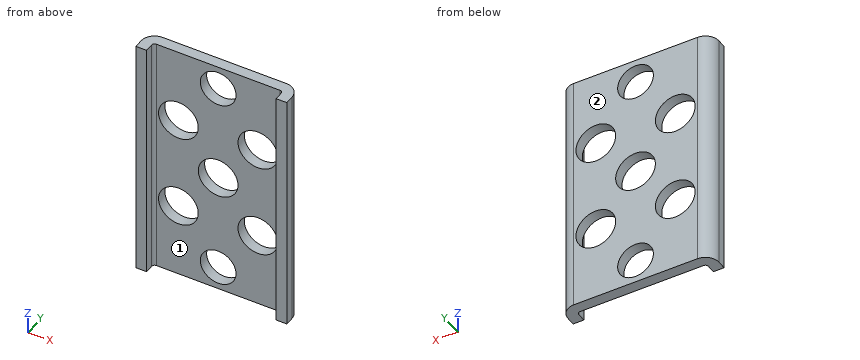
```python
from build123d import *

# Parameters (mm, degrees)
SKETCH1_W                      = 37.995749454
SKETCH1_H                      = 62
BOSS_EXTRUDE1_DEPTH            = 5.594860996
SKETCH2_W                      = 32.595749454
SKETCH2_H                      = 2.894860996
CUT_EXTRUDE1_DEPTH             = 66.086263633
F_10_0_10_DIAMETER_HOLE1_D     = 10
F_10_0_10_DIAMETER_HOLE1_DEPTH = 5.594860996
F_9_0_9_DIAMETER_HOLE1_D       = 9
F_9_0_9_DIAMETER_HOLE1_DEPTH   = 5.594860996
FILLET1_R                      = 0.7366
FILLET2_R                      = 3.4366


with BuildPart() as part:
    # Sketch1 → Boss-Extrude1 (new body)
    with BuildSketch(Plane(origin=(0, 0, 0), x_dir=(1, 0, 0), z_dir=(0, 1, 0))):
        with Locations((0, 45)):
            Rectangle(SKETCH1_W, SKETCH1_H)
    extrude(amount=-BOSS_EXTRUDE1_DEPTH)

    # Sketch2 → Cut-Extrude1 (cut, through all)
    with BuildSketch(Plane(origin=(0, 0, -76), x_dir=(-1, 0, 0), z_dir=(0, 0, -1))):
        with Locations((0, -4.147430498)):
            Rectangle(SKETCH2_W, SKETCH2_H)
    extrude(amount=-CUT_EXTRUDE1_DEPTH, mode=Mode.SUBTRACT)

    # Ø10.0 (10) Diameter Hole1
    with Locations(Plane(origin=(0, 0, 0), x_dir=(1, 0, 0), z_dir=(0, 1, 0))):
        with Locations((0, 45), (-10, 57), (-10, 33), (10, 33), (10, 57)):
            Hole(F_10_0_10_DIAMETER_HOLE1_D / 2, depth=F_10_0_10_DIAMETER_HOLE1_DEPTH)

    # Ø9.0 (9) Diameter Hole1
    with Locations(Plane(origin=(0, 0, 0), x_dir=(1, 0, 0), z_dir=(0, 1, 0))):
        with Locations((0, 70), (0, 20)):
            Hole(F_9_0_9_DIAMETER_HOLE1_D / 2, depth=F_9_0_9_DIAMETER_HOLE1_DEPTH)

    # Fillet1
    fillet1_edges = [part.edges().sort_by_distance(p)[0] for p in [
        (16.297874727, -2.7, -45),
        (-16.297874727, -2.7, -45),
    ]]
    fillet(fillet1_edges, radius=FILLET1_R)

    # Fillet2
    fillet2_edges = [part.edges().sort_by_distance(p)[0] for p in [
        (18.997874727, 0, -45),
        (-18.997874727, 0, -45),
    ]]
    fillet(fillet2_edges, radius=FILLET2_R)


solid = part.part
```
For this review, take the finished solid that the model builds, in its own axes (mm). Face numbers are marked on the shaded views. A direction names the side the tool comes from. Round coordinates to 2 decimals unless told otherwise and drop trailing zeros. Order: outer loops, then holes, each group sorted by start corner. A loop starts at its lowest first (then second) coordinate and runs counter-clockwise, first axis right, second up. Notation, with made-up numbers: (-7.75, -0.75) -> (4.25, -0.75) arc R27 ccw to (4.25, 21.25) -> close; hole circle Ø1 at (77, 14). An arc over 180 degrees is marked (long way). Use a Markdown table: item, result.
Item 1: Machinability: for the marked faces 1 and 2, which of the approach directions +Z, -Z, +X, -X, +Y, -Y give a long, thin tool a straight path to every point of the face, cutting with its end or side? Answer none if there is none.
Resolved:
| item | result |
|---|---|
| face 1 | +Z, -Z, -Y |
| face 2 | +Z, -Z, +X, -X, +Y |
Item 2: For line 1 along Z through (x, y) = (-10, -2); line 2 along Z through (x, y) = (0, -1.45); line 3 along X through (y, z) = (-4.55, -45.5), list the stretches that pass through material, from the lowest coordinate up. Write a range as [from, to].
Resolved:
| item | result |
|---|---|
| line 1 | z = [-76, -62], [-52, -38], [-28, -14] |
| line 2 | z = [-76, -74.5], [-65.5, -50], [-40, -24.5], [-15.5, -14] |
| line 3 | x = [-19, -16.3], [16.3, 19] |
Item 3: Take a section at C-C (z = -33). State the section outline as (x, y) points, plus the area to 3 significant figures.
Resolved:
| item | result |
|---|---|
| outline | (-19, -5.59) -> (-16.3, -5.59) -> (-16.3, -3.44) arc R0.74 cw to (-15.56, -2.7) -> (-15, -2.7) -> (-15, 0) -> (-15.56, 0) arc R3.44 ccw to (-19, -3.44) -> close; (-5, -2.7) -> (5, -2.7) -> (5, 0) -> (-5, 0) -> close; (15, -2.7) -> (15.56, -2.7) arc R0.74 cw to (16.3, -3.44) -> (16.3, -5.59) -> (19, -5.59) -> (19, -3.44) arc R3.44 ccw to (15.56, 0) -> (15, 0) -> close |
| area | 59.4 mm² |
Item 4: Take a section at B-B (z = -70). State the section outline as (x, y) points, plus the area to 3 significant figures.
Resolved:
| item | result |
|---|---|
| outline | (-19, -5.59) -> (-16.3, -5.59) -> (-16.3, -3.44) arc R0.74 cw to (-15.56, -2.7) -> (-4.5, -2.7) -> (-4.5, 0) -> (-15.56, 0) arc R3.44 ccw to (-19, -3.44) -> close; (4.5, -2.7) -> (15.56, -2.7) arc R0.74 cw to (16.3, -3.44) -> (16.3, -5.59) -> (19, -5.59) -> (19, -3.44) arc R3.44 ccw to (15.56, 0) -> (4.5, 0) -> close |
| area | 89.1 mm² |
Item 5: Take a section at A-A (x = 7). State the section outline as (y, z) points, plus the area to 3 significant figures.
Resolved:
| item | result |
|---|---|
| outline | (-2.7, -76) -> (0, -76) -> (0, -61) -> (-2.7, -61) -> close; (-2.7, -53) -> (0, -53) -> (0, -37) -> (-2.7, -37) -> close; (-2.7, -29) -> (0, -29) -> (0, -14) -> (-2.7, -14) -> close |
| area | 124 mm² |
Item 6: For pin 1 (1.5 mm diameter, centred on x = -12.5, y = -5, fed in from +Z); pin 2 (15.5 mm diameter, centred on x = 0, z = -47, fed in from -Y); pin 3 (13 mm diameter, centred on x = 10, z = -33, fed in from -Y); pin 4 (3 mm diameter, centred on x = -14.5, z = -56, fed in from -Y), all flat-tipped, find the tip position at first contact; note any pin that passes through.
Resolved:
| item | result |
|---|---|
| pin 1 | passes through |
| pin 2 | stops at y = -2.7 |
| pin 3 | stops at y = -5.59 |
| pin 4 | stops at y = -2.84 |
Item 7: Take a section at D-D (y = -1.6). State the section outline as (x, z) points, plus the area to 3 significant figures.
Resolved:
| item | result |
|---|---|
| outline | (-18.47, -76) -> (18.47, -76) -> (18.47, -14) -> (-18.47, -14) -> close; hole circle Ø10 at (-10, -57); hole circle Ø10 at (-10, -33); hole circle Ø10 at (0, -45); hole circle Ø9 at (0, -70); hole circle Ø9 at (0, -20); hole circle Ø10 at (10, -57); hole circle Ø10 at (10, -33) |
| area | 1,770 mm² |
